from build123d import *

# Parameters (mm, degrees)
SKETCH_1_W          = 700
SKETCH_1_H          = 900
EXTRUDE_1_DEPTH     = 2
CUT_EXTRUDE_1_DEPTH = 10
SKETCH_3_R          = 40
CUT_EXTRUDE_2_DEPTH = 10


with BuildPart() as part:
    # 草图1 → 凸台-拉伸1 (new body)
    with BuildSketch(Plane.XY):
        Rectangle(SKETCH_1_W, SKETCH_1_H)
    extrude(amount=EXTRUDE_1_DEPTH)

    # 草图2 → 切除-拉伸1 (cut)
    with BuildSketch(Plane.XY.offset(2)):
        with BuildLine():
            Line((-337.75, 180), (-337.75, 170))
            ThreePointArc((-337.75, 170), (-340, 167.75), (-342.25, 170))
            Line((-342.25, 170), (-342.25, 180))
            ThreePointArc((-342.25, 180), (-340, 182.25), (-337.75, 180))
        make_face()
        with BuildLine():
            Line((-342.25, -5), (-342.25, 5))
            ThreePointArc((-342.25, 5), (-340, 7.25), (-337.75, 5))
            Line((-337.75, 5), (-337.75, -5))
            ThreePointArc((-337.75, -5), (-340, -7.25), (-342.25, -5))
        make_face()
        with BuildLine():
            Line((337.75, 170), (337.75, 180))
            ThreePointArc((337.75, 180), (340, 182.25), (342.25, 180))
            Line((342.25, 180), (342.25, 170))
            ThreePointArc((342.25, 170), (340, 167.75), (337.75, 170))
        make_face()
        with BuildLine():
            Line((342.25, -5), (342.25, 5))
            ThreePointArc((342.25, 5), (340, 7.25), (337.75, 5))
            Line((337.75, 5), (337.75, -5))
            ThreePointArc((337.75, -5), (340, -7.25), (342.25, -5))
        make_face()
        with BuildLine():
            Line((-342.25, 360), (-342.25, 350))
            ThreePointArc((-342.25, 350), (-340, 347.75), (-337.75, 350))
            Line((-337.75, 350), (-337.75, 360))
            ThreePointArc((-337.75, 360), (-340, 362.25), (-342.25, 360))
        make_face()
        with BuildLine():
            Line((337.75, -170), (337.75, -180))
            ThreePointArc((337.75, -180), (340, -182.25), (342.25, -180))
            Line((342.25, -180), (342.25, -170))
            ThreePointArc((342.25, -170), (340, -167.75), (337.75, -170))
        make_face()
        with BuildLine():
            Line((342.25, 360), (342.25, 350))
            ThreePointArc((342.25, 350), (340, 347.75), (337.75, 350))
            Line((337.75, 350), (337.75, 360))
            ThreePointArc((337.75, 360), (340, 362.25), (342.25, 360))
        make_face()
        with BuildLine():
            Line((342.25, -360), (342.25, -350))
            ThreePointArc((342.25, -350), (340, -347.75), (337.75, -350))
            Line((337.75, -350), (337.75, -360))
            ThreePointArc((337.75, -360), (340, -362.25), (342.25, -360))
        make_face()
        with BuildLine():
            Line((-342.25, -360), (-342.25, -350))
            ThreePointArc((-342.25, -350), (-340, -347.75), (-337.75, -350))
            Line((-337.75, -350), (-337.75, -360))
            ThreePointArc((-337.75, -360), (-340, -362.25), (-342.25, -360))
        make_face()
        with BuildLine():
            Line((-337.75, -170), (-337.75, -180))
            ThreePointArc((-337.75, -180), (-340, -182.25), (-342.25, -180))
            Line((-342.25, -180), (-342.25, -170))
            ThreePointArc((-342.25, -170), (-340, -167.75), (-337.75, -170))
        make_face()
    extrude(amount=-CUT_EXTRUDE_1_DEPTH, mode=Mode.SUBTRACT)

    # 草图3 → 切除-拉伸2 (cut)
    with BuildSketch(Plane.XY.offset(2)):
        with Locations((-100, 300)):
            Circle(SKETCH_3_R)
        with Locations((100, 300)):
            Circle(SKETCH_3_R)
    extrude(amount=-CUT_EXTRUDE_2_DEPTH, mode=Mode.SUBTRACT)


solid = part.part
Can you work these out from the model? Positions are in its coordinate system, mm. Coordinates: 2 decimals unless noted, no trailing zeros. Order: outer loops, then holes, each group sorted by start corner. A loop starts at its lowest first (then second) coordinate and runs counter-clockwise, first axis right, second up. Notation, with made-up numbers: (-14, 46) - (27, 46) arc R13 ccw to (27, 59) - close; hole circle Ø7 at (72.5, -11.75). An arc over 180 degrees is marked (long way). Answer as a JSON object with one key per item and string values. Group by question number.
Q1. We'd pull the mould along X, two halves only. Please class faces 1 (the face through (121.5, 333.73, 1.01)), 2 (the face through (-5, 6, 2)), 3 (the face through (-78.5, 333.73, 1.01)): +X half, -X half, draft (parallel to the pull), parting line (faces both ways), or undercut.
Q2. Imagine slicing it at A-A (x = -97.5). Please give me the cut outline in (y, z).
Q3. Imagine slicing it at B-B (z = 0.7). Give the number of separate pieces and of enclosed holes in the cut face, and give its area (3 significant figures).
Q4. I need wall thicknesses on line 1 (Y direction, x = -100, z = 1.5); line 2 (X direction, y = 361.5, z = 0.9); line 3 (Y direction, x = -121, z = 0.6). Which ranges of each line are inside material? Lowest first, please. Write a range as from..to.
Determined:
{
 "1": {"face 1": "undercut", "face 2": "draft", "face 3": "undercut"},
 "2": {"outline": "(-450, 0) - (260.08, 0) - (260.08, 2) - (-450, 2) - close; (339.92, 0) - (450, 0) - (450, 2) - (339.92, 2) - close"},
 "3": {"separate pieces": "1", "enclosed holes": "12", "area": "619,000 mm2"},
 "4": {"line 1": "y = -450..260, 340..450", "line 2": "x = -350..-341.68, -338.32..338.32, 341.68..350", "line 3": "y = -450..265.96, 334.04..450"}
}
